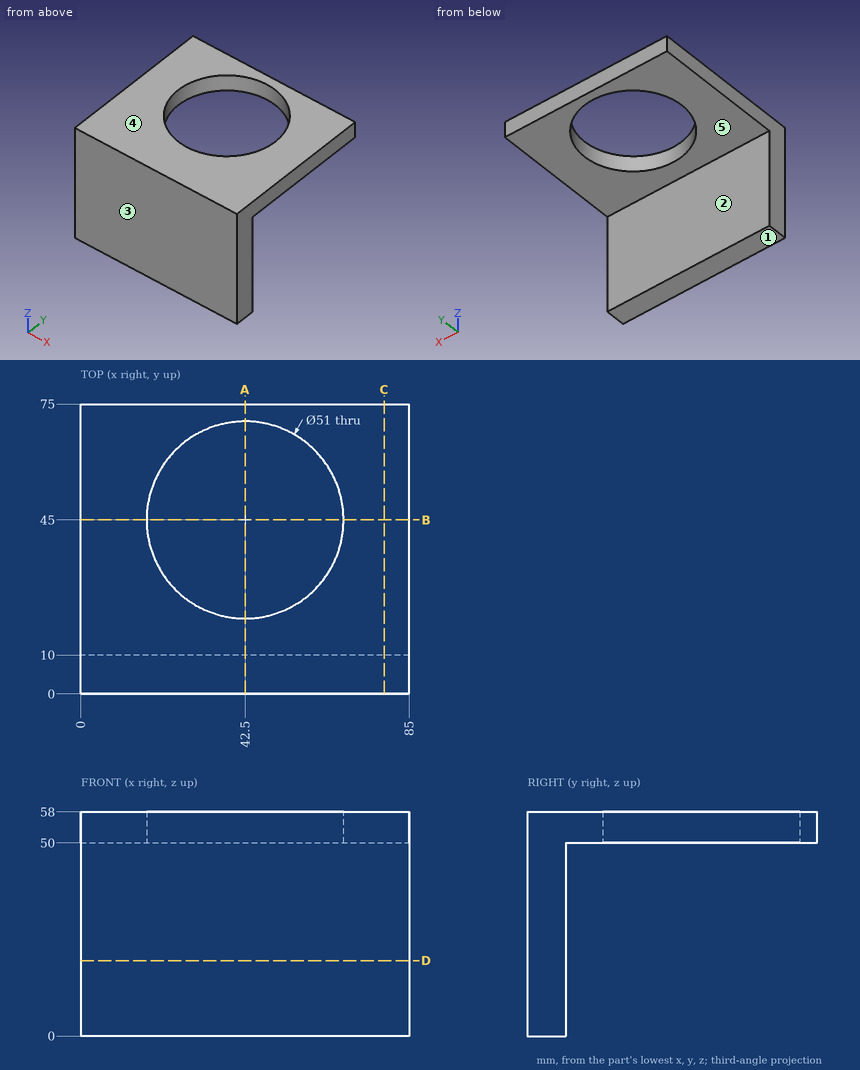
The drawing under review shows one solid part. Ordinate dimensions are in mm from its lowest x, y, z. A direction names the side the tool comes from. Round coordinates to 2 decimals unless told otherwise and drop trailing zeros. Order: outer loops, then holes, each group sorted by start corner. A loop starts at its lowest first (then second) coordinate and runs counter-clockwise, first axis right, second up. Notation, with made-up numbers: (8.25, 63) -> (49.25, 63) arc R20 cw to (49.25, 89) -> close; hole circle Ø4 at (59, -17). An arc over 180 degrees is marked (long way). Return JSON: item names as keys, results as strings.
1. Take a section at D-D (z = 19.5). Write out the cut boundary in (x, y), then the cut area to 3 significant figures.
Answer block:
{"outline": "(0, 0) -> (85, 0) -> (85, 10) -> (0, 10) -> close", "area": "850 mm²"}
2. Insertion check: P1, Ø8, axis at x = 12, y = 67, coming from the -Z side; P2, Ø1, axis at x = 11, z = 43.5, coming from the +Y side. Each pin has a flat end and moves straight along its axis. Give the tip position at first contact, or say it passes through.
Answer block:
{"P1": "stops at z = 50", "P2": "stops at y = 10"}
3. The part is to be moulded in two halves that separate along Y. For the marked faces 1, 2 and 3, say which applies: +Y half, -Y half, draft (parallel to the pull), parting line (faces both ways), or undercut.
Answer block:
{"face 1": "draft", "face 2": "+Y half", "face 3": "-Y half"}
4. For the marked faces 4 and 5, list the 3-axis set-ups (+Z, -Z, +X, -X, +Y, -Y) from which the entire face can be reached by the end or side of a thin tool; tool diameter is ignored.
Answer block:
{"face 4": "+Z, +X, -X, +Y, -Y", "face 5": "-Z, +X, -X, +Y"}
5. Take a section at C-C (x = 78.5). Write out the cut boundary in (y, z), then the cut area to 3 significant figures.
Answer block:
{"outline": "(0, 0) -> (10, 0) -> (10, 50) -> (75, 50) -> (75, 58) -> (0, 58) -> close", "area": "1,100 mm²"}
6. Take a section at A-A (x = 42.5). Write out the cut boundary in (y, z).
Answer block:
{"outline": "(0, 0) -> (10, 0) -> (10, 50) -> (19.5, 50) -> (19.5, 58) -> (0, 58) -> close; (70.5, 50) -> (75, 50) -> (75, 58) -> (70.5, 58) -> close"}
7. Take a section at B-B (y = 45). Write out the cut boundary in (x, z), then the cut area to 3 significant figures.
Answer block:
{"outline": "(0, 50) -> (17, 50) -> (17, 58) -> (0, 58) -> close; (68, 50) -> (85, 50) -> (85, 58) -> (68, 58) -> close", "area": "272 mm²"}
8. For L1, parallel to Y at x = 42.5, z = 52.5; L2, parallel to Z at x = 60, y = 18; L3, parallel to Y at x = 28, z = 49.5, list the stretches that pass through material, from the lowest coordinate up. Write a range as [from, to].
Answer block:
{"L1": "y = [0, 19.5], [70.5, 75]", "L2": "z = [50, 58]", "L3": "y = [0, 10]"}
